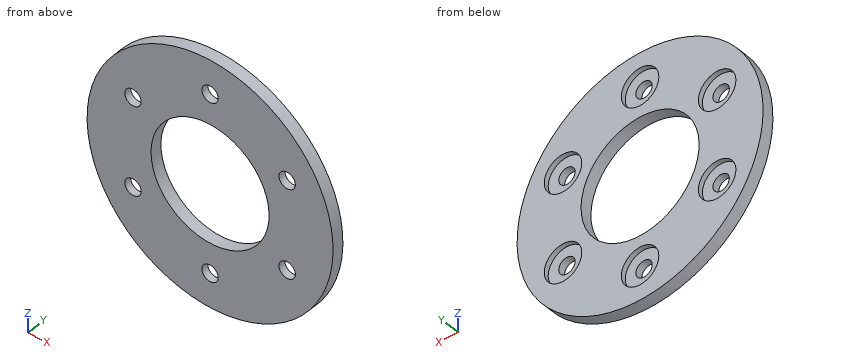
from build123d import *

# Parameters (mm, degrees)
SKETCH1_R           = 26.25
SKETCH1_R_2         = 12.6
BOSS_EXTRUDE1_DEPTH = 4
SKETCH2_R           = 35
SKETCH2_R_2         = 14.25
CUT_EXTRUDE1_DEPTH  = 1.5
SKETCH4_R           = 1.75
CUT_EXTRUDE2_DEPTH  = 10
CIRPATTERN1_COUNT   = 6
SKETCH5_R           = 4
CUT_EXTRUDE3_DEPTH  = 1
CIRPATTERN2_COUNT   = 6
CHAMFER1_SIZE       = 0.5
SKETCH6_R           = 14.25
CUT_EXTRUDE4_DEPTH  = 1.5


with BuildPart() as part:
    # Sketch1 → Boss-Extrude1 (new body)
    with BuildSketch(Plane(origin=(0, 0, 0), x_dir=(1, 0, 0), z_dir=(0, 1, 0))):
        with Locations(Location((0, 0, 0), (0, 0, 270))):
            Circle(SKETCH1_R)
        with Locations(Location((0, 0, 0), (0, 0, 270))):
            Circle(SKETCH1_R_2, mode=Mode.SUBTRACT)
    extrude(amount=BOSS_EXTRUDE1_DEPTH)

    # Sketch2 → Cut-Extrude1 (cut)
    with BuildSketch(Plane(origin=(0, 4, 0), x_dir=(1, 0, 0), z_dir=(0, 1, 0))):
        Circle(SKETCH2_R)
        with Locations(Location((0, 0, 0), (0, 0, 270))):
            Circle(SKETCH2_R_2, mode=Mode.SUBTRACT)
    extrude(amount=-CUT_EXTRUDE1_DEPTH, mode=Mode.SUBTRACT)

    # Sketch4 → Cut-Extrude2 (cut)
    with BuildSketch(Plane(origin=(0, 2.5, 0), x_dir=(1, 0, 0), z_dir=(0, 1, 0))):
        with Locations(Location((0, 19, 0), (0, 0, 270))):
            Circle(SKETCH4_R)
    cut_extrude2 = extrude(amount=-CUT_EXTRUDE2_DEPTH, mode=Mode.SUBTRACT)

    # CirPattern1: Cut-Extrude2 ×6 about axis
    cirpattern1_axis = Axis((0, 0, 0), (0, 1, 0))
    for i in range(1, CIRPATTERN1_COUNT):
        add(cut_extrude2.rotate(cirpattern1_axis, i * 360 / CIRPATTERN1_COUNT), mode=Mode.SUBTRACT)

    # Sketch5 → Cut-Extrude3 (cut)
    with BuildSketch(Plane(origin=(0, 2.5, 0), x_dir=(1, 0, 0), z_dir=(0, 1, 0))):
        with Locations(Location((0, 19, 0), (0, 0, 270))):
            Circle(SKETCH5_R)
    cut_extrude3 = extrude(amount=-CUT_EXTRUDE3_DEPTH, mode=Mode.SUBTRACT)

    # CirPattern2: Cut-Extrude3 ×6 about axis
    cirpattern2_axis = Axis((0, 0, 0), (0, 1, 0))
    for i in range(1, CIRPATTERN2_COUNT):
        add(cut_extrude3.rotate(cirpattern2_axis, i * 360 / CIRPATTERN2_COUNT), mode=Mode.SUBTRACT)

    # Chamfer1
    chamfer1_edges = [part.edges().sort_by_distance(p)[0] for p in [
        (0, 4, -14.25),
    ]]
    chamfer(chamfer1_edges, length=CHAMFER1_SIZE)

    # Sketch6 → Cut-Extrude4 (cut)
    with BuildSketch(Plane(origin=(0, 4, 0), x_dir=(1, 0, 0), z_dir=(0, 1, 0))):
        Circle(SKETCH6_R)
    extrude(amount=-CUT_EXTRUDE4_DEPTH, mode=Mode.SUBTRACT)


solid = part.part
Can you work these out from the model? Positions are in its coordinate system, mm. Give positions to 0.01 mm unless a question says otherwise; leave off trailing zeros. Order: outer loops, then holes, each group sorted by start corner. A loop starts at its lowest first (then second) coordinate and runs counter-clockwise, first axis right, second up. Notation, with made-up numbers: M 82.25,51 L 137.25,51 A24 cw 137.25,84 Z; hole C 16,75 d5. An arc over 180 degrees is marked long. One line per item, written item: value.
Item 1: If we section it at A-A on z = 0: Write out the boundary of the cut face in (x, y), and give its area (4 significant figures).
Verdict:
outline: M -26.25,0 L -12.6,0 L -12.6,2.5 L -26.25,2.5 Z; M 12.6,0 L 26.25,0 L 26.25,2.5 L 12.6,2.5 Z
area: 68.25 mm2
Item 2: Please list where these lines run through material, in increasing order: line 1 (Z direction, x = 17.5, y = 0.65); line 2 (Z direction, x = -19, y = 1.6); line 3 (X direction, y = 2.05, z = 9.5).
Verdict:
line 1: -19.57 to -10.9, -8.1 to 8.1, 10.9 to 19.57
line 2: -18.11 to -12.59, -6.41 to 6.41, 12.59 to 18.11
line 3: -24.47 to -20.45, -12.45 to -8.28, 8.28 to 12.45, 20.45 to 24.47
Item 3: If we section it at B-B on x = 0: Write out the boundary of the cut face in (y, z).
Verdict:
outline: M 0,-26.25 L 2.5,-26.25 L 2.5,-23 L 1.5,-23 L 1.5,-20.75 L 0,-20.75 Z; M 0,-17.25 L 1.5,-17.25 L 1.5,-15 L 2.5,-15 L 2.5,-12.6 L 0,-12.6 Z; M 0,12.6 L 2.5,12.6 L 2.5,15 L 1.5,15 L 1.5,17.25 L 0,17.25 Z; M 0,20.75 L 1.5,20.75 L 1.5,23 L 2.5,23 L 2.5,26.25 L 0,26.25 Z
Item 4: If we section it at C-C on y = 0.9: Write out the boundary of the cut face in (x, z) (3 decimals).
Verdict:
outline: C 0,0 d52.5; hole C -16.454,-9.5 d3.5; hole C -16.454,9.5 d3.5; hole C 0,0 d25.2; hole C 0,-19 d3.5; hole C 0,19 d3.5; hole C 16.454,-9.5 d3.5; hole C 16.454,9.5 d3.5
Item 5: For pin 1 (1 mm diameter, centred on y = 0.5, z = 4, fed in from -X); pin 2 (5.5 mm diameter, centred on x = 0, z = -19, fed in from +Y); pin 3 (1 mm diameter, centred on x = -4, y = 2, fed in from +Z), each with a flat end and sliding along its axis, tell me the tip position at first contact or that it passes through.
Verdict:
pin 1: x = -26.02
pin 2: y = 1.5
pin 3: z = 26.02
Item 6: If we section it at D-D on x = -10: Write out the boundary of the cut face in (y, z).
Verdict:
outline: M 0,-24.27 L 2.5,-24.27 L 2.5,-7.67 L 0,-7.67 Z; M 0,7.67 L 2.5,7.67 L 2.5,24.27 L 0,24.27 Z
